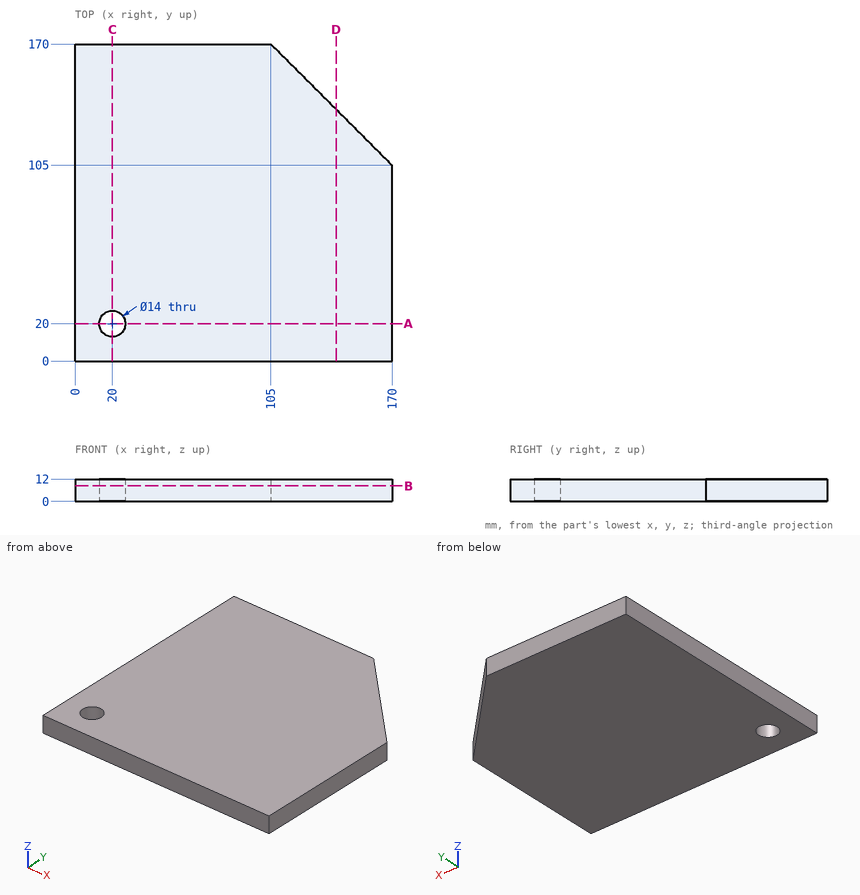
Source: three-view drawing plus pictorial views. Frame: mm from the lowest corner of the part. Coordinates: 2 decimals unless noted, no trailing zeros. Loops run counter-clockwise (first coordinate to the right, second up) from the corner with the lowest first, then second, coordinate; pieces in that order, holes last. Notation, with made-up numbers: (-0.5, 72) -> (25.5, 72) arc R16 cw to (25.5, 84) -> close; hole circle Ø1 at (18.5, 2). An arc over 180 degrees is marked (long way). Answer in a Markdown table with one row per item. Add a question column.
Q1. Section A-A on y = 20. Return the cut outline in (x, z), and give its area (3 significant figures).
Q2. Ray query, line 1 along Y through (x, z) = (20, 9.25); line 2 along Y through (x, z) = (24.5, 11.25); line 3 along X through (y, z) = (157, 5). Return the intervals inside material, ascending.
Q3. Section D-D on x = 140. Return the cut outline in (y, z), and give its area (3 significant figures).
Q4. Contact query for a flat-ended pin moving along its axis: pin 1 Ø1.5 at (y, z) = (133, 4) entering from +X. Output: stop coordinate, or through.
Q5. Section B-B on z = 8.25. Return the cut outline in (x, y), and give its area (3 significant figures).
Computed values:
| question | item | result |
|---|---|---|
| 1 | outline | (0, 0) -> (13, 0) -> (13, 12) -> (0, 12) -> close; (27, 0) -> (170, 0) -> (170, 12) -> (27, 12) -> close |
| 1 | area | 1,870 mm^2 |
| 2 | line 1 | y = 0 to 13, 27 to 170 |
| 2 | line 2 | y = 0 to 14.64, 25.36 to 170 |
| 2 | line 3 | x = 0 to 118 |
| 3 | outline | (0, 0) -> (135, 0) -> (135, 12) -> (0, 12) -> close |
| 3 | area | 1,620 mm^2 |
| 4 | pin 1 | stops at x = 142.75 |
| 5 | outline | (0, 0) -> (170, 0) -> (170, 105) -> (105, 170) -> (0, 170) -> close; hole circle Ø14 at (20, 20) |
| 5 | area | 26,600 mm^2 |
